Verification items for the finished model (mm, model axes). Face numbers are marked on the shaded views. A direction names the side the tool comes from. Coordinates: 2 decimals unless noted, no trailing zeros. Order: outer loops, then holes, each group sorted by start corner. A loop starts at its lowest first (then second) coordinate and runs counter-clockwise, first axis right, second up. Notation, with made-up numbers: M 21.25,0.5 L 65.25,0.5 A25 ccw 65.25,38.5 Z; hole C -24.5,-18 d9. An arc over 180 degrees is marked long. Return JSON: item names as keys, results as strings. Group by question number.
1. Section check C-C, the plane y = 133. Record the cut outline in (x, z).
2. Section check B-B, the plane z = -29. Record the cut outline in (x, y).
3. Section check D-D, the plane z = -18.5. Record the cut outline in (x, y), plus the area to 3 significant figures.
4. Set-up check for the marked faces 1 and 2: record each of +Z, -Z, +X, -X, +Y, -Y from which the full face is reachable in a straight line by a thin tool's end or side.
5. Section check A-A, the plane x = 200. Record the cut outline in (y, z).
6. Gauge pin test, flat end, axial feed: pin 1 (1.5 mm diameter, centred on x = 211.5, y = 144.5, fed in from -Z). Record the tip position at first contact, or that the pin passes through.
7. Material ranges on line 1 along Z through (x, y) = (191, 136.5); line 2 along Y through (x, z) = (192.5, -50.5); line 3 along X through (y, z) = (117, -50), recorded low to high.
```python
from build123d import *

# Parameters (mm, degrees)
GB_T706_2008_63_X_40_X_6_1_DEPTH = 40
CUT_EXTRUDE_1_DEPTH              = 10


with BuildPart() as part:
    # Sketch1 → 热轧不等边角钢gb∕t706-2008 63 X 40 X 6(1) (new body)
    with BuildSketch(Plane(origin=(220, 114, 0), x_dir=(0, 1, 0), z_dir=(-1, 0, 0))):
        with BuildLine():
            Line((0, 0), (0, 63))
            Line((0, 63), (3.666666667, 63))
            ThreePointArc((3.666666667, 63), (5.316582489, 62.316582489), (6, 60.666666667))
            Line((6, 60.666666667), (6, 13))
            ThreePointArc((6, 13), (8.050252532, 8.050252532), (13, 6))
            Line((13, 6), (37.666666667, 6))
            ThreePointArc((37.666666667, 6), (39.316582489, 5.316582489), (40, 3.666666667))
            Line((40, 3.666666667), (40, 0))
            Line((40, 0), (0, 0))
        make_face()
    extrude(amount=GB_T706_2008_63_X_40_X_6_1_DEPTH)

    # 草图2 → 切除-拉伸1 (cut)
    with BuildSketch(Plane(origin=(0, 120, 0), x_dir=(1, 0, 0), z_dir=(0, 1, 0))):
        with BuildLine():
            Line((206.25, 45), (206.25, 20))
            ThreePointArc((206.25, 20), (200, 13.75), (193.75, 20))
            Line((193.75, 20), (193.75, 45))
            ThreePointArc((193.75, 45), (200, 51.25), (206.25, 45))
        make_face()
    extrude(amount=-CUT_EXTRUDE_1_DEPTH, mode=Mode.SUBTRACT)


solid = part.part
```
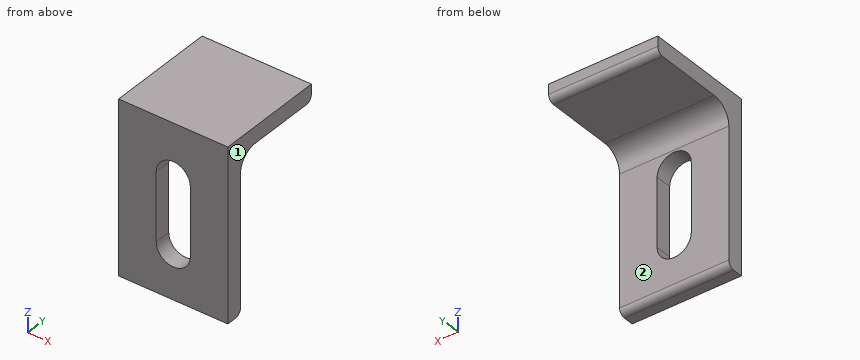
Answers follow:
{
 "1": {"outline": "M 180,-6 L 220,-6 L 220,0 L 180,0 Z"},
 "2": {"outline": "M 180,114 L 193.75,114 L 193.75,120 L 180,120 Z; M 206.25,114 L 220,114 L 220,120 L 206.25,120 Z"},
 "3": {"outline": "M 180,114 L 193.93,114 L 193.93,120 L 180,120 Z; M 206.07,114 L 220,114 L 220,120 L 206.07,120 Z", "area": "167 mm^2"},
 "4": {"face 1": "+Z, -Z, +X, +Y, -Y", "face 2": "-Z, +X, -X, +Y"},
 "5": {"outline": "M 114,-63 L 117.67,-63 A2.33 ccw 120,-60.67 L 120,-51.25 L 114,-51.25 Z; M 114,-13.75 L 120,-13.75 L 120,-13 A7 cw 127,-6 L 151.67,-6 A2.33 ccw 154,-3.67 L 154,0 L 114,0 Z"},
 "6": {"pin 1": "z = -6"},
 "7": {"line 1": "-6 to 0", "line 2": "114 to 120", "line 3": "180 to 196.25, 203.75 to 220"}
}
